Read the model definition and answer for the solid it produces. Units are mm, in the model's axes. Round coordinates to 2 decimals unless told otherwise and drop trailing zeros. Loops run counter-clockwise (first coordinate to the right, second up) from the corner with the lowest first, then second, coordinate; pieces in that order, holes last. Notation, with made-up numbers: (0.5, -16) -> (30.5, -16) arc R8 cw to (30.5, -12) -> close; hole circle Ø1 at (-5, 77). An arc over 180 degrees is marked (long way). Put each result on its own line as item: value.
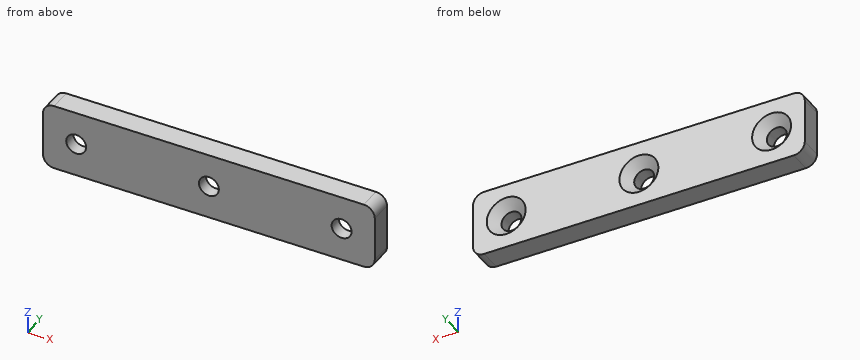
from build123d import *

# Parameters (mm, degrees)
SKETCH1_W                                  = 150
SKETCH1_H                                  = 30
BOSS_EXTRUDE1_DEPTH                        = 10
FILLET1_R                                  = 5
SOCKET_BUTTON_HEAD_SCREW_HOLE1_D           = 9
SOCKET_BUTTON_HEAD_SCREW_HOLE1_DEPTH       = 19.75
SOCKET_BUTTON_HEAD_SCREW_HOLE1_CSINK_D     = 17.6
SOCKET_BUTTON_HEAD_SCREW_HOLE1_CSINK_ANGLE = 90
SOCKET_BUTTON_HEAD_SCREW_HOLE1_TIP         = 2.703872786


with BuildPart() as part:
    # Sketch1 → Boss-Extrude1 (new body)
    with BuildSketch(Plane(origin=(0, 0, 0), x_dir=(1, 0, 0), z_dir=(0, 1, 0))):
        with Locations((75, 15)):
            Rectangle(SKETCH1_W, SKETCH1_H)
    extrude(amount=BOSS_EXTRUDE1_DEPTH)

    # Fillet1
    fillet1_edges = [part.edges().sort_by_distance(p)[0] for p in [
        (0, 5, -30),
        (150, 5, -30),
        (150, 5, 0),
        (0, 5, 0),
    ]]
    fillet(fillet1_edges, radius=FILLET1_R)

    # Socket Button Head Screw Hole1
    with Locations(Plane(origin=(0, 10, 0), x_dir=(1, 0, 0), z_dir=(0, 1, 0))):
        with Locations((75, 15), (15, 15), (135, 15)):
            CounterSinkHole(SOCKET_BUTTON_HEAD_SCREW_HOLE1_D / 2, SOCKET_BUTTON_HEAD_SCREW_HOLE1_CSINK_D / 2, depth=SOCKET_BUTTON_HEAD_SCREW_HOLE1_DEPTH, counter_sink_angle=SOCKET_BUTTON_HEAD_SCREW_HOLE1_CSINK_ANGLE)
            with Locations((0, 0, -(SOCKET_BUTTON_HEAD_SCREW_HOLE1_DEPTH + SOCKET_BUTTON_HEAD_SCREW_HOLE1_TIP / 2))):  # 118° drill point
                Cone(0, SOCKET_BUTTON_HEAD_SCREW_HOLE1_D / 2, SOCKET_BUTTON_HEAD_SCREW_HOLE1_TIP, mode=Mode.SUBTRACT)


solid = part.part
Item 1: The part is cut by section A-A (y = 2). Determine the outline of the cut face in (x, z).
Derived:
outline: (0, -25) arc R5 ccw to (5, -30) -> (145, -30) arc R5 ccw to (150, -25) -> (150, -5) arc R5 ccw to (145, 0) -> (5, 0) arc R5 ccw to (0, -5) -> close; hole circle Ø9 at (15, -15); hole circle Ø9 at (75, -15); hole circle Ø9 at (135, -15)
Item 2: The part is cut by section C-C (z = -15). Determine the outline of the cut face in (x, y), then the cut area to 3 significant figures.
Derived:
outline: (0, 0) -> (10.5, 0) -> (10.5, 5.7) -> (6.2, 10) -> (0, 10) -> close; (19.5, 0) -> (70.5, 0) -> (70.5, 5.7) -> (66.2, 10) -> (23.8, 10) -> (19.5, 5.7) -> close; (79.5, 0) -> (130.5, 0) -> (130.5, 5.7) -> (126.2, 10) -> (83.8, 10) -> (79.5, 5.7) -> close; (139.5, 0) -> (150, 0) -> (150, 10) -> (143.8, 10) -> (139.5, 5.7) -> close
area: 1,170 mm^2
Item 3: The part is cut by section B-B (x = 75). Determine the outline of the cut face in (y, z), then the cut area to 3 significant figures.
Derived:
outline: (0, -30) -> (10, -30) -> (10, -23.8) -> (5.7, -19.5) -> (0, -19.5) -> close; (0, -10.5) -> (5.7, -10.5) -> (10, -6.2) -> (10, 0) -> (0, 0) -> close
area: 192 mm^2
Item 4: Find the intervals of material crossed by line 1 along X through (y, z) = (3, -14.5); line 2 along Z through (x, y) = (135, 1.95); line 3 along X through (y, z) = (2.25, -14), in increasing order.
Derived:
line 1: x = 0 to 10.53, 19.47 to 70.53, 79.47 to 130.53, 139.47 to 150
line 2: z = -30 to -19.5, -10.5 to 0
line 3: x = 0 to 10.61, 19.39 to 70.61, 79.39 to 130.61, 139.39 to 150
Item 5: Flat-ended cylindrical pins translate along their axes: pin 1 Ø10.5 at (x, z) = (75, -15) entering from +Y; pin 2 Ø5.5 at (x, z) = (15, -15) entering from -Y. Find the tip coordinate at first contact, or state that the pin passes through.
Derived:
pin 1: stops at y = 6.45
pin 2: passes through
